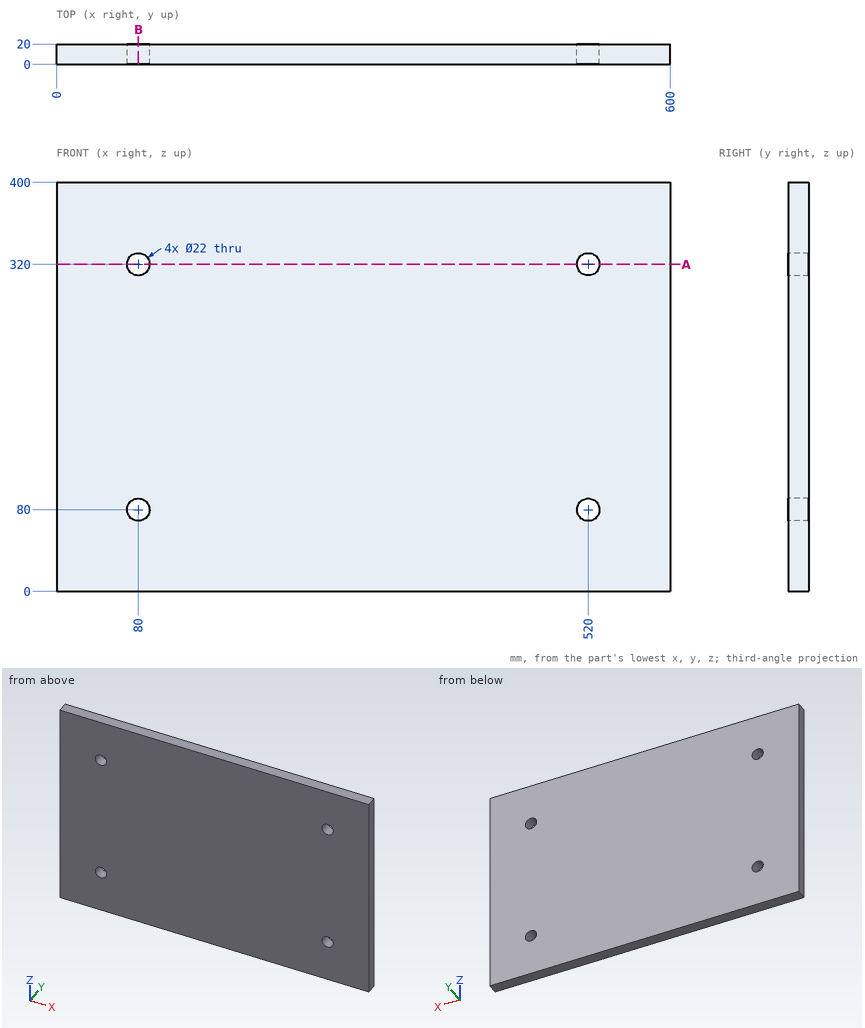
Source: three-view drawing plus pictorial views. Frame: mm from the lowest corner of the part. Coordinates: 2 decimals unless noted, no trailing zeros. Order: outer loops, then holes, each group sorted by start corner. A loop starts at its lowest first (then second) coordinate and runs counter-clockwise, first axis right, second up.
Item 1: Material intervals for line 1 (X direction, y = 11.5, z = 320); line 2 (X direction, y = 2.5, z = 314.5), sorted ascending.
Output values:
line 1: x = 0 to 69, 91 to 509, 531 to 600
line 2: x = 0 to 70.47, 89.53 to 510.47, 529.53 to 600
Item 2: Cut plane B-B (x = 80). Return loops of the section in (y, z), plus the area to 3 significant figures.
Output values:
outline: (0, 0) - (20, 0) - (20, 69) - (0, 69) - close; (0, 91) - (20, 91) - (20, 309) - (0, 309) - close; (0, 331) - (20, 331) - (20, 400) - (0, 400) - close
area: 7,120 mm2
Item 3: Cut plane A-A (z = 320). Return loops of the section in (x, y), plus the area to 3 significant figures.
Output values:
outline: (0, 0) - (69, 0) - (69, 20) - (0, 20) - close; (91, 0) - (509, 0) - (509, 20) - (91, 20) - close; (531, 0) - (600, 0) - (600, 20) - (531, 20) - close
area: 11,100 mm2
